Verification items for this drawing (mm, ordinates from the low corner). A direction names the side the tool comes from. Round coordinates to 2 decimals unless told otherwise and drop trailing zeros. Loops run counter-clockwise (first coordinate to the right, second up) from the corner with the lowest first, then second, coordinate; pieces in that order, holes last. Notation, with made-up numbers: (61.5, 58.5) -> (114.5, 58.5) arc R23 ccw to (114.5, 77.5) -> close; hole circle Ø11 at (-10, 15). An arc over 180 degrees is marked (long way). Use a Markdown table: item, result. Add a question column.
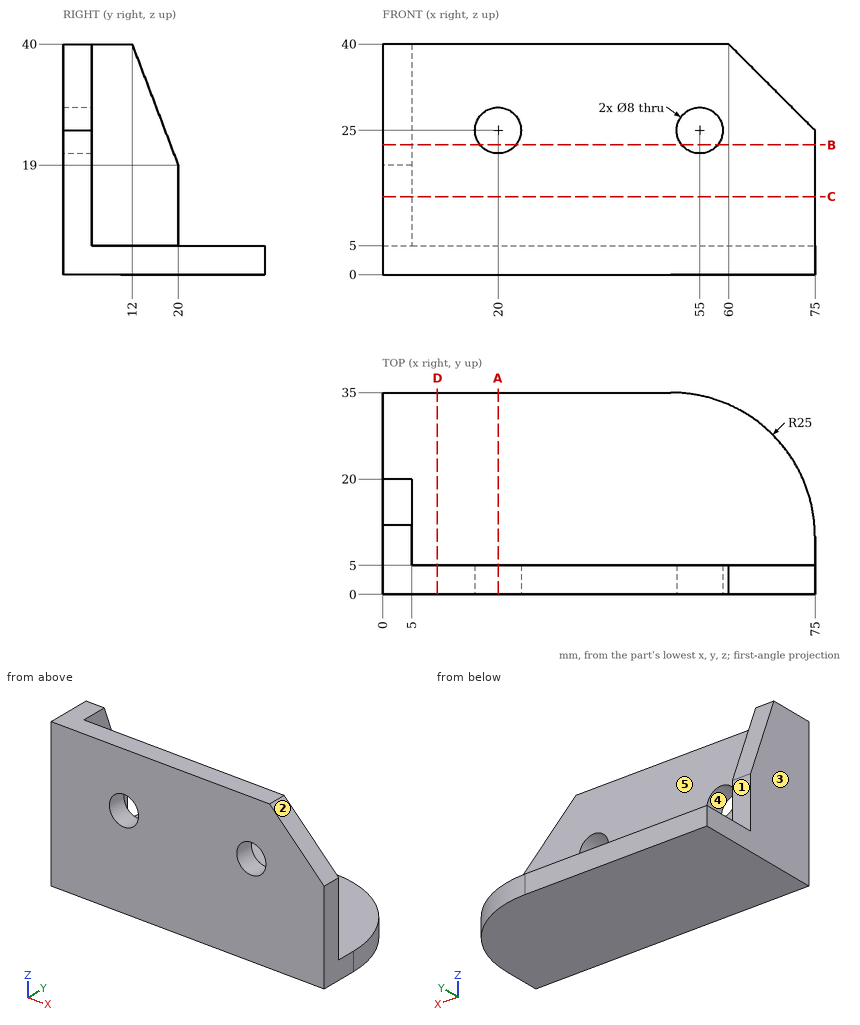
1) Thickness scan on line 1 (X direction, y = 3, z = 25); line 2 (Z direction, x = 58, y = 11). Record the ranges inside material, lowest first.
2) Sectioned sample at A-A on x = 20. Enter the section's corners in (y, z).
3) Sectioned sample at C-C on z = 13.5. Enter the section's corners in (x, y).
4) Access from +Z, -Z, +X, -X, +Y, -Y to the whole of each face (thin tool, end or side, straight path). Record for the marked faces 1 and 2.
5) Sectioned sample at D-D on x = 9.5. Enter the section's corners in (y, z).
6) Go/stop test with flat-tipped pins: pin 1 (12 mm diameter, centred on x = 65.5, z = 17.5, fed in from -Y); pin 2 (2 mm diameter, centred on x = 32.5, y = 30.5, fed in from +Z); pin 3 (8 mm diameter, centred on y = 19, z = 4.5, fed in from +X); pin 4 (8 mm diameter, centred on x = 11.5, z = 15.5, fed in from +Y). Record where each tip stops, or that it passes through.
7) Release check for a two-part mould opening along X. For the marked faces 3, 4 and 5 record: released by +X, released by -X, zero draft, split by the parting line, or undercut.
8) Sectioned sample at B-B on z = 22.5. Enter the section's corners in (x, y), then the cut area to 3 significant figures.
Geometry results:
| question | item | result |
|---|---|---|
| 1 | line 1 | 0 to 16, 24 to 51, 59 to 75 |
| 1 | line 2 | 0 to 5 |
| 2 | outline | (0, 0) -> (35, 0) -> (35, 5) -> (5, 5) -> (5, 21) -> (0, 21) -> close; (0, 29) -> (5, 29) -> (5, 40) -> (0, 40) -> close |
| 3 | outline | (0, 0) -> (75, 0) -> (75, 5) -> (5, 5) -> (5, 20) -> (0, 20) -> close |
| 4 | face 1 | +Z, +X, -X, +Y |
| 4 | face 2 | +Z, +X, +Y, -Y |
| 5 | outline | (0, 0) -> (35, 0) -> (35, 5) -> (5, 5) -> (5, 40) -> (0, 40) -> close |
| 6 | pin 1 | y = 0 |
| 6 | pin 2 | z = 5 |
| 6 | pin 3 | x = 74.49 |
| 6 | pin 4 | y = 5 |
| 7 | face 3 | released by -X |
| 7 | face 4 | undercut |
| 7 | face 5 | zero draft |
| 8 | outline | (0, 0) -> (16.88, 0) -> (16.88, 5) -> (5, 5) -> (5, 18.67) -> (0, 18.67) -> close; (23.12, 0) -> (51.88, 0) -> (51.88, 5) -> (23.12, 5) -> close; (58.12, 0) -> (75, 0) -> (75, 5) -> (58.12, 5) -> close |
| 8 | area | 381 mm^2 |
